For this review, take the finished solid that the model builds, in its own axes (mm). A direction names the side the tool comes from. Round coordinates to 2 decimals unless told otherwise and drop trailing zeros. Order: outer loops, then holes, each group sorted by start corner. A loop starts at its lowest first (then second) coordinate and runs counter-clockwise, first axis right, second up. Notation, with made-up numbers: (30.5, 72) -> (78.5, 72) arc R18 ccw to (78.5, 87) -> close; hole circle Ø1 at (-26.75, -28.5). An arc over 180 degrees is marked (long way). Answer in a Markdown table with one row per item.
```python
from build123d import *

# Parameters (mm, degrees)
SKETCH_1_W             = 217
SKETCH_1_H             = 196.5
SKETCH_1_R             = 74
EXTRUDE_1_DEPTH        = 12
SKETCH_2_R             = 91.25
CUT_EXTRUDE_1_DEPTH    = 2
CUT_EXTRUDE_START      = -2
SKETCH_3_R             = 91.25
CUT_EXTRUDE_2_DEPTH    = 2
SKETCH_4_W             = 39.75
SKETCH_4_H             = 120
CUT_EXTRUDE_3_DEPTH    = 2
HOLE_WIZARD_M6_1_D     = 6.6
HOLE_WIZARD_M8_1_D     = 6.8
HOLE_WIZARD_M8_1_DEPTH = 19.75
HOLE_WIZARD_M8_1_TIP   = 2.042926105
HOLE_WIZARD_M8_2_D     = 6.8
HOLE_WIZARD_M8_2_DEPTH = 19.75
HOLE_WIZARD_M8_2_TIP   = 2.042926105


with BuildPart() as part:
    # 草图1 → 凸台-拉伸1 (new body)
    with BuildSketch(Plane.XY):
        Rectangle(SKETCH_1_W, SKETCH_1_H)
        Circle(SKETCH_1_R, mode=Mode.SUBTRACT)
    extrude(amount=EXTRUDE_1_DEPTH)

    # 草图2 → 切除-拉伸1 (cut)
    with BuildSketch(Plane(origin=(0, 0, 0), x_dir=(-1, 0, 0), z_dir=(0, 0, -1))):
        Circle(SKETCH_2_R)
    extrude(amount=-CUT_EXTRUDE_1_DEPTH, mode=Mode.SUBTRACT)

    # 草图3 → 切除-拉伸2 (cut)
    with BuildSketch(Plane.XY.offset(12).offset(CUT_EXTRUDE_START)):
        with Locations(Location((0, 0, 0), (0, 0, 180))):
            Circle(SKETCH_3_R)
    extrude(amount=CUT_EXTRUDE_2_DEPTH, mode=Mode.SUBTRACT)

    # 草图4 → 切除-拉伸3 (cut)
    with BuildSketch(Plane.XY.offset(12)):
        with Locations((-88.625, 0)):
            Rectangle(SKETCH_4_W, SKETCH_4_H)
    extrude(amount=-CUT_EXTRUDE_3_DEPTH, mode=Mode.SUBTRACT)

    # M6 间隙孔1 (through all)
    with Locations(Plane(origin=(0, 0, 2), x_dir=(-1, 0, 0), z_dir=(0, 0, -1))):
        with Locations((0, 84), (42, 72.746133918), (72.746133918, 42), (84, 0), (72.746133918, -42), (42, -72.746133918), (0, -84), (-42, -72.746133918), (-72.746133918, -42), (-84, 0), (-72.746133918, 42), (-42, 72.746133918)):
            Hole(HOLE_WIZARD_M6_1_D / 2)

    # M8 螺纹孔1
    with Locations(Plane(origin=(0, -98.25, 0), x_dir=(-1, 0, 0), z_dir=(0, -1, 0))):
        with Locations((-95, -6), (-40, -6), (40, -6), (95, -6)):
            Hole(HOLE_WIZARD_M8_1_D / 2, depth=HOLE_WIZARD_M8_1_DEPTH)
            with Locations((0, 0, -(HOLE_WIZARD_M8_1_DEPTH + HOLE_WIZARD_M8_1_TIP / 2))):  # 118° drill point
                Cone(0, HOLE_WIZARD_M8_1_D / 2, HOLE_WIZARD_M8_1_TIP, mode=Mode.SUBTRACT)

    # M8 螺纹孔2
    with Locations(Plane(origin=(0, 98.25, 0), x_dir=(1, 0, 0), z_dir=(0, 1, 0))):
        with Locations((-95, -6), (-40, -6), (40, -6), (95, -6)):
            Hole(HOLE_WIZARD_M8_2_D / 2, depth=HOLE_WIZARD_M8_2_DEPTH)
            with Locations((0, 0, -(HOLE_WIZARD_M8_2_DEPTH + HOLE_WIZARD_M8_2_TIP / 2))):  # 118° drill point
                Cone(0, HOLE_WIZARD_M8_2_D / 2, HOLE_WIZARD_M8_2_TIP, mode=Mode.SUBTRACT)


solid = part.part
```
Q1. Take a section at D-D, the plane x = -84. Write out the cut boundary in (y, z).
Answer key:
| item | result |
|---|---|
| outline | (-98.25, 0) -> (-35.64, 0) -> (-35.64, 2) -> (-3.3, 2) -> (-3.3, 10) -> (-60, 10) -> (-60, 12) -> (-98.25, 12) -> close; (3.3, 2) -> (35.64, 2) -> (35.64, 0) -> (98.25, 0) -> (98.25, 12) -> (60, 12) -> (60, 10) -> (3.3, 10) -> close |
Q2. Take a section at C-C, the plane y = 6.5. Write out the cut boundary in (x, z).
Answer key:
| item | result |
|---|---|
| outline | (-108.5, 0) -> (-91.02, 0) -> (-91.02, 2) -> (-73.71, 2) -> (-73.71, 10) -> (-108.5, 10) -> close; (73.71, 2) -> (91.02, 2) -> (91.02, 0) -> (108.5, 0) -> (108.5, 12) -> (91.02, 12) -> (91.02, 10) -> (73.71, 10) -> close |
Q3. Take a section at B-B, the plane y = -42. Write out the cut boundary in (x, z).
Answer key:
| item | result |
|---|---|
| outline | (-108.5, 0) -> (-81.01, 0) -> (-81.01, 2) -> (-76.05, 2) -> (-76.05, 10) -> (-108.5, 10) -> close; (-69.45, 2) -> (-60.93, 2) -> (-60.93, 10) -> (-69.45, 10) -> close; (60.93, 2) -> (69.45, 2) -> (69.45, 10) -> (60.93, 10) -> close; (76.05, 2) -> (81.01, 2) -> (81.01, 0) -> (108.5, 0) -> (108.5, 12) -> (81.01, 12) -> (81.01, 10) -> (76.05, 10) -> close |
Q4. Tool access review of faces 5 (the face through (-91.6, 88.2, 5.9)), 6 (the face through (-76, 7, 10)), 7 (the face through (95.59, -76.81, 5.97)): name each direction out of +Z, -Z, +X, -X, +Y, -Y from which nothing blocks a thin tool from reaching the whole face with its end or side.
Answer key:
| item | result |
|---|---|
| face 5 | +Y |
| face 6 | +Z |
| face 7 | -Y |
Q5. The part is to be moulded in two halves that separate along Y. For faces 1 (the face through (-95.59, 76.81, 5.97)), 2 (the face through (-6, -74, 2)), 3 (the face through (74.52, 44.783, 6.056)), 4 (the face through (-108.5, -1, 6)), say which applies: +Y half, -Y half, draft (parallel to the pull), parting line (faces both ways), or undercut.
Answer key:
| item | result |
|---|---|
| face 1 | +Y half |
| face 2 | undercut |
| face 3 | undercut |
| face 4 | draft |
Q6. Take a section at A-A, the plane x = -33. Write out the cut boundary in (y, z), then the cut area to 3 significant figures.
Answer key:
| item | result |
|---|---|
| outline | (-98.25, 0) -> (-85.07, 0) -> (-85.07, 2) -> (-66.23, 2) -> (-66.23, 10) -> (-85.07, 10) -> (-85.07, 12) -> (-98.25, 12) -> close; (66.23, 2) -> (85.07, 2) -> (85.07, 0) -> (98.25, 0) -> (98.25, 12) -> (85.07, 12) -> (85.07, 10) -> (66.23, 10) -> close |
| area | 618 mm^2 |
Q7. Clearance check with flat-ended pins moving along their axes: pin 1 Ø6 at (x, z) = (-95, 6) entering from -Y; pin 2 Ø8 at (x, y) = (60.5, 38) entering from +Z; pin 3 Ø4 at (x, y) = (42, -72.75) entering from -Z; pin 4 Ø5.5 at (x, z) = (95, 6) entering from +Y. State where each tip first meets the part, or that it passes through.
Answer key:
| item | result |
|---|---|
| pin 1 | stops at y = -78.26 |
| pin 2 | stops at z = 10 |
| pin 3 | passes through |
| pin 4 | stops at y = 78.11 |
Q8. To check wall thickness, follow probe 1 along Y at (x, z) = (-42, 6.5); probe 2 along X at (y, z) = (-58.5, 6); probe 3 along Z at (x, y) = (-17, -72.5). State the ranges of each line that lie inside material, in increasing order.
Answer key:
| item | result |
|---|---|
| probe 1 | y = -77.7 to -76.05, -69.45 to -60.93, 60.93 to 69.45, 76.05 to 77.7 |
| probe 2 | x = -108.5 to -45.32, 45.32 to 108.5 |
| probe 3 | z = 2 to 10 |
